The model under review builds one solid part; all positions refer to its coordinate system, in mm. Coordinates: 2 decimals unless noted, no trailing zeros. Write each loop counter-clockwise with the first axis right and the second up, starting at its lowest first coordinate (ties: lowest second). Pieces come first, ordered by that corner, then holes. Notation, with made-up numbers: (-37, 76.5) - (6, 76.5) arc R30 cw to (6, 112.5) - close; hole circle Ø4 at (31.5, 79.5). An arc over 180 degrees is marked (long way). Put each result on its own line as item: value.
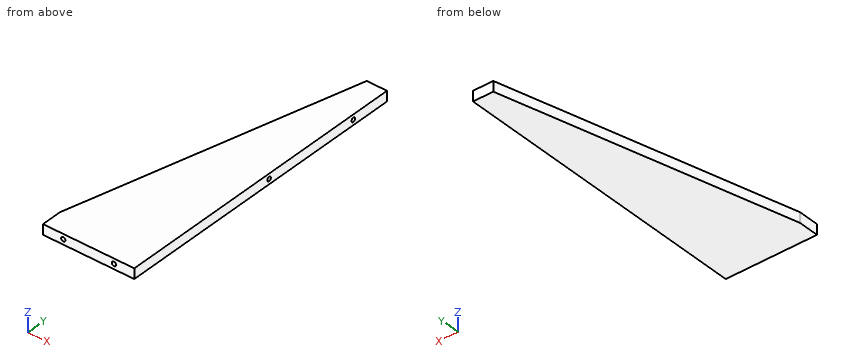
from build123d import *

# Parameters (mm, degrees)
SKETCH_1_W             = 90
SKETCH_1_H             = 300
EXTRUDE_1_DEPTH        = 10
CUT_EXTRUDE_1_REACH    = 158.924
HOLE_WIZARD_M5_1_D     = 4.2
HOLE_WIZARD_M5_1_DEPTH = 14.4
HOLE_WIZARD_M5_1_TIP   = 1.2618073
HOLE_WIZARD_M5_2_D     = 4.2
HOLE_WIZARD_M5_2_DEPTH = 14.4
HOLE_WIZARD_M5_2_TIP   = 1.2618073


with BuildPart() as part:
    # 草图1 → 凸台-拉伸1 (new body)
    with BuildSketch(Plane.XY):
        Rectangle(SKETCH_1_W, SKETCH_1_H)
    extrude(amount=EXTRUDE_1_DEPTH)

    # 草图2 → 切除-拉伸1 (cut, up to next)
    with BuildSketch(Plane.XY.offset(10), mode=Mode.PRIVATE) as cut_extrude_1_sk1:
        Polygon((25, 150), (-45, 150), (-45, -130), align=None)
    cut_extrude_1_tool1 = extrude(cut_extrude_1_sk1.sketch, amount=-CUT_EXTRUDE_1_REACH, mode=Mode.PRIVATE) & part.part
    add(cut_extrude_1_tool1.solids().sort_by_distance((-21.666667, 56.666667, 10))[0], mode=Mode.SUBTRACT)

    # M5 螺纹孔1
    with Locations(Plane(origin=(0, -150, 0), x_dir=(-1, 0, 0), z_dir=(0, -1, 0))):
        with Locations((-25, -5), (25, -5)):
            Hole(HOLE_WIZARD_M5_1_D / 2, depth=HOLE_WIZARD_M5_1_DEPTH)
            with Locations((0, 0, -(HOLE_WIZARD_M5_1_DEPTH + HOLE_WIZARD_M5_1_TIP / 2))):  # 118° drill point
                Cone(0, HOLE_WIZARD_M5_1_D / 2, HOLE_WIZARD_M5_1_TIP, mode=Mode.SUBTRACT)

    # M5 螺纹孔2
    with Locations(Plane(origin=(45, 0, 0), x_dir=(0, 0, -1), z_dir=(1, 0, 0))):
        with Locations((-5, 110), (-5, 10)):
            Hole(HOLE_WIZARD_M5_2_D / 2, depth=HOLE_WIZARD_M5_2_DEPTH)
            with Locations((0, 0, -(HOLE_WIZARD_M5_2_DEPTH + HOLE_WIZARD_M5_2_TIP / 2))):  # 118° drill point
                Cone(0, HOLE_WIZARD_M5_2_D / 2, HOLE_WIZARD_M5_2_TIP, mode=Mode.SUBTRACT)


solid = part.part
1. Consider section B-B on x = -5. State the section outline as (y, z) points.
Determined:
outline: (-150, 0) - (30, 0) - (30, 10) - (-150, 10) - close
2. For pin 1 Ø4 at (y, z) = (110, 5) entering from -X, flat-tipped, find the tip position at first contact; note if it passes through.
Determined:
pin 1: stops at x = 14.5
3. To check wall thickness, follow probe 1 along Y at (x, z) = (40.5, 5); probe 2 along Y at (x, z) = (31, 5.5); probe 3 along Z at (x, y) = (39.75, 110). State the ranges of each line that lie inside material, in increasing order.
Determined:
probe 1: y = -150 to 7.9, 12.1 to 107.9, 112.1 to 150
probe 2: y = -150 to 7.96, 12.04 to 107.96, 112.04 to 150
probe 3: z = 0 to 2.9, 7.1 to 10
4. Consider section A-A on y = 75. State the section outline as (x, z) points.
Determined:
outline: (6.25, 0) - (45, 0) - (45, 10) - (6.25, 10) - close
